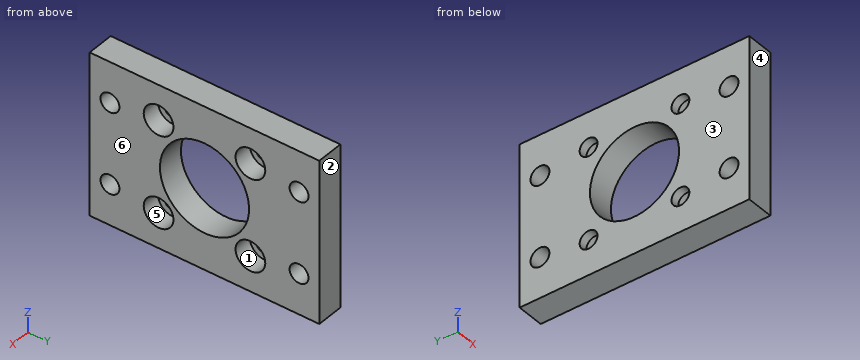
from build123d import *

# Parameters (mm, degrees)
SKETCH_1_W                = 60
SKETCH_1_H                = 85
EXTRUDE_1_DEPTH           = 10
HOLE_WIZARD_1_D           = 6.6
HOLE_WIZARD_1_CBORE_D     = 11
HOLE_WIZARD_1_CBORE_DEPTH = 6.8
HOLE_WIZARD_7_0_7_1_D     = 7
SKETCH_6_R                = 16.5
CUT_EXTRUDE_1_DEPTH       = 53.974050251


with BuildPart() as part:
    # 草图1 → 凸台-拉伸1 (new body)
    with BuildSketch(Plane(origin=(0, 0, 0), x_dir=(0, 0, -1), z_dir=(1, 0, 0))):
        Rectangle(SKETCH_1_W, SKETCH_1_H)
    extrude(amount=EXTRUDE_1_DEPTH)

    # 打孔尺寸(%根据)内六角圆柱头螺钉的类型1 (through all)
    with Locations(Plane(origin=(10, 0, 0), x_dir=(0, 0, -1), z_dir=(1, 0, 0))):
        with Locations((-17, 17), (17, 17), (-17, -17), (17, -17)):
            CounterBoreHole(HOLE_WIZARD_1_D / 2, HOLE_WIZARD_1_CBORE_D / 2, HOLE_WIZARD_1_CBORE_DEPTH)

    # Ø7.0 (7) 直径孔1 (through all)
    with Locations(Plane.ZY):
        with Locations((-15, 35), (15, 35), (-15, -35), (15, -35)):
            Hole(HOLE_WIZARD_7_0_7_1_D / 2)

    # 草图6 → 切除-拉伸1 (cut, through all)
    with BuildSketch(Plane.ZY):
        Circle(SKETCH_6_R)
    extrude(amount=-CUT_EXTRUDE_1_DEPTH, mode=Mode.SUBTRACT)


solid = part.part
The model under review builds one solid part; all positions refer to its coordinate system, in mm. Face numbers are marked on the shaded views. A direction names the side the tool comes from. Round coordinates to 2 decimals unless told otherwise and drop trailing zeros. Order: outer loops, then holes, each group sorted by start corner. A loop starts at its lowest first (then second) coordinate and runs counter-clockwise, first axis right, second up. Notation, with made-up numbers: (53, -35.75) -> (97, -35.75) arc R15 ccw to (97, -18.75) -> close; hole circle Ø3 at (-24.75, 85.5). An arc over 180 degrees is marked (long way). Write item = value, one per line. Start each with the question number.
Item 1: Consider section A-A on y = -35. Write out the cut boundary in (x, z).
Item 2: For line 1 along Y through (x, z) = (1.8, -17); line 2 along Z through (x, y) = (5, -20); line 3 along Y through (x, z) = (7, 17), list the stretches that pass through material, from the lowest coordinate up.
Item 3: Mouldability with a two-part tool opening along Y and no side actions: class the marked faces 1, 2, 3 and 4 as released by +Y, released by -Y, zero draft, split by the parting line, or undercut.
Item 4: Consider section B-B on z = 0. Write out the cut boundary in (x, y), plus the area to 3 significant figures.
Item 5: For the marked faces 5 and 6, list the 3-axis set-ups (+Z, -Z, +X, -X, +Y, -Y) from which the entire face can be reached by the end or side of a thin tool; tool diameter is ignored.
Item 6: Consider section D-D on y = 0. Write out the cut boundary in (x, z), plus the area to 3 significant figures.
Item 7: Clearance check with flat-ended pins moving along their axes: pin 1 Ø6.5 at (y, z) = (-17, -17) entering from +X; pin 2 Ø3.5 at (y, z) = (-16.5, 19.5) entering from +X. State where each tip first meets the part, or that it passes through.
Item 8: Consider section C-C on x = 1.25. Count the separate pieces of the cut face and the enclosed holes in it, plus the area to 3 significant figures.
Conclusion:
q1.outline = (0, -30) -> (10, -30) -> (10, -18.5) -> (0, -18.5) -> close; (0, -11.5) -> (10, -11.5) -> (10, 11.5) -> (0, 11.5) -> close; (0, 18.5) -> (10, 18.5) -> (10, 30) -> (0, 30) -> close
q2.line_1 = -42.5 to -37.87, -32.13 to -20.3, -13.7 to 13.7, 20.3 to 32.13, 37.87 to 42.5
q2.line_2 = -30 to -21.61, -12.39 to 12.39, 21.61 to 30
q2.line_3 = -42.5 to -37.87, -32.13 to -22.5, -11.5 to 11.5, 22.5 to 32.13, 37.87 to 42.5
q3.face_1 = undercut
q3.face_2 = released by +Y
q3.face_3 = zero draft
q3.face_4 = released by -Y
q4.outline = (0, -42.5) -> (10, -42.5) -> (10, -16.5) -> (0, -16.5) -> close; (0, 16.5) -> (10, 16.5) -> (10, 42.5) -> (0, 42.5) -> close
q4.area = 520 mm2
q5.face_5 = +X
q5.face_6 = +Z, -Z, +X, +Y, -Y
q6.outline = (0, -30) -> (10, -30) -> (10, -16.5) -> (0, -16.5) -> close; (0, 16.5) -> (10, 16.5) -> (10, 30) -> (0, 30) -> close
q6.area = 270 mm2
q7.pin_1 = through
q7.pin_2 = 3.2
q8.separate_pieces = 1
q8.enclosed_holes = 9
q8.area = 3,950 mm2
